Verification items for the finished model (mm, model axes). A direction names the side the tool comes from. Give positions to 0.01 mm unless a question says otherwise; leave off trailing zeros. Write each loop counter-clockwise with the first axis right and the second up, starting at its lowest first coordinate (ties: lowest second). Pieces come first, ordered by that corner, then holes. Notation, with made-up numbers: (13.25, -21) - (21.25, -21) arc R4 ccw to (21.25, -14) - close; hole circle Ø4 at (60.5, 33.5). An arc over 180 degrees is marked (long way). Answer as a JSON object with one key per item and string values. Group by question number.
Item 1: Sectioned sample at D-D, the plane y = 98.5. Record the boundary of the cut face in (x, z), and give its area (3 significant figures).
Item 2: Draft check along X on faces 5 (the face through (52, 207, -25)), 6 (the face through (-17.367, 90.897, -2.1)), 7 (the face through (100, 93, 1)). Enter one of: +X half, -X half, draft (parallel to the pull), parting line (faces both ways), or undercut.
Item 3: Sectioned sample at B-B, the plane y = 50.5. Record the boundary of the cut face in (x, z).
Item 4: Sectioned sample at C-C, the plane x = 55. Record the boundary of the cut face in (y, z), and give its area (3 significant figures).
Item 5: Tool access check on faces 1 (the face through (-94, 95, -65)), 2 (the face through (94, 95, 65)), 3 (the face through (52, 208, 25)), 4 (the face through (79, 57, -40)). Record the directions out of +Z, -Z, +X, -X, +Y, -Y that give a thin tool (end or side, any length) a straight path to the whole face; none if there is none.
Item 6: Go/stop test with flat-tipped pins: pin 1 (7.5 mm diameter, centred on y = 204, z = 51.5, fed in from -X); pin 2 (12.5 mm diameter, centred on x = -44.5, y = 204.5, fed in from +Z); pin 3 (23 mm diameter, centred on x = -87.5, y = 65, fed in from +Z); pin 4 (2 mm diameter, centred on x = -3.5, z = 119, fed in from +Y). Record where each tip stops, or that it passes through.
Item 7: Sectioned sample at A-A, the plane z = -46.5. Record the boundary of the cut face in (x, y), and give its area (3 significant figures).
Item 8: Scan lines: line 1 along Y through (x, z) = (43.5, -29.5); line 2 along Y through (x, z) = (89.5, -36); line 3 along Z through (x, y) = (-91.5, 95). Record each from-to range of solid material in increasing order. Write a range as [from, to].
```python
from build123d import *

# Parameters (mm, degrees)
INCLINED_BASE_BLOCK_DEPTH           = 100
FRONT_NOTCH_CUT_DEPTH               = 285.429253067
FRONT_NOTCH_CUT_DEPTH_BACK          = 285.429253067
FRONT_NOTCH_SKETCH_OUTSIDE_W        = 286.474
FRONT_NOTCH_SKETCH_OUTSIDE_H        = 306.474
TOP_RECESS_CUT_DEPTH                = 285.429253067
TOP_RECESS_CUT_DEPTH_BACK           = 285.429253067
FRONT_FRAME_BOSS_DEPTH              = 65
TOP_CROSS_SLOT_CUT_80X80_DEPTH      = 334.016516107
TOP_CROSS_SLOT_CUT_80X80_DEPTH_BACK = 334.016516107
TOP_CROSS_SLOT_SKETCH_W             = 80
TOP_CROSS_SLOT_SKETCH_H             = 80


with BuildPart() as part:
    # Base Profile Sketch → Inclined Base Block (new, symmetric)
    with BuildSketch(Plane(origin=(0, 0, 0), x_dir=(0, 0, -1), z_dir=(1, 0, 0))):
        Polygon((-150, 0), (-80, 220), (-25, 220), (-25, 195), (25, 195), (25, 220), (80, 220), (150, 0), align=None)
    extrude(amount=INCLINED_BASE_BLOCK_DEPTH, both=True)

    # Front Notch Sketch outside → Front Notch Cut (cut, two sides: drawn at the far end of the back side and taken through both)
    with BuildSketch(Plane.XY.offset(-FRONT_NOTCH_CUT_DEPTH_BACK)):
        with Locations((0, 110)):
            Rectangle(FRONT_NOTCH_SKETCH_OUTSIDE_W, FRONT_NOTCH_SKETCH_OUTSIDE_H)
        Polygon((-100, 0), (-65, 220), (-35, 220), (-35, 195), (35, 195), (35, 220), (65, 220), (100, 0), align=None, mode=Mode.SUBTRACT)
    extrude(amount=FRONT_NOTCH_CUT_DEPTH + FRONT_NOTCH_CUT_DEPTH_BACK, mode=Mode.SUBTRACT)

    # Top Recess Sketch → Top Recess Cut (cut, two sides: drawn at the far end of the back side and taken through both)
    with BuildSketch(Plane.XY.offset(-TOP_RECESS_CUT_DEPTH_BACK)):
        Polygon((-100, 0), (0, 110), (100, 0), align=None)
    extrude(amount=TOP_RECESS_CUT_DEPTH + TOP_RECESS_CUT_DEPTH_BACK, mode=Mode.SUBTRACT)

    # Front Frame Sketch → Front Frame Boss (add, symmetric)
    with BuildSketch(Plane.XY):
        Polygon((100, 0), (100, 130), (79.318181818, 130), align=None)
    front_frame_boss = extrude(amount=FRONT_FRAME_BOSS_DEPTH, both=True)

    # Front Frame Mirror: Front Frame Boss across plane
    add(front_frame_boss.mirror(Plane(origin=(0, 0, 0), x_dir=(0, 0, 1), z_dir=(1, 0, 0))))

    # Top Cross Slot Sketch → Top Cross Slot Cut 80x80 (cut, two sides: drawn at the far end of the back side and taken through both)
    with BuildSketch(Plane(origin=(100, 0, 0), x_dir=(0, 0, -1), z_dir=(1, 0, 0)).offset(-TOP_CROSS_SLOT_CUT_80X80_DEPTH_BACK)):
        with Locations((0, 40)):
            Rectangle(TOP_CROSS_SLOT_SKETCH_W, TOP_CROSS_SLOT_SKETCH_H)
    extrude(amount=TOP_CROSS_SLOT_CUT_80X80_DEPTH + TOP_CROSS_SLOT_CUT_80X80_DEPTH_BACK, mode=Mode.SUBTRACT)


solid = part.part
```
Geometry check:
{
 "1": {"outline": "(-100, -65) - (-84.33, -65) - (-84.33, -118.66) - (-10.45, -118.66) - (-10.45, 118.66) - (-84.33, 118.66) - (-84.33, 65) - (-100, 65) - close; (10.45, -118.66) - (84.33, -118.66) - (84.33, -65) - (100, -65) - (100, 65) - (84.33, 65) - (84.33, 118.66) - (10.45, 118.66) - close", "area": "39,100 mm^2"},
 "2": {"face 5": "draft", "face 6": "undercut", "face 7": "+X half"},
 "3": {"outline": "(-100, -65) - (-91.97, -65) - (-91.97, -133.93) - (-54.09, -133.93) - (-54.09, -40) - (-100, -40) - close; (-100, 40) - (-54.09, 40) - (-54.09, 133.93) - (-91.97, 133.93) - (-91.97, 65) - (-100, 65) - close; (54.09, -133.93) - (91.97, -133.93) - (91.97, -65) - (100, -65) - (100, -40) - (54.09, -40) - close; (54.09, 40) - (100, 40) - (100, 65) - (91.97, 65) - (91.97, 133.93) - (54.09, 133.93) - close"},
 "4": {"outline": "(49.5, -134.25) - (220, -80) - (220, -25) - (195, -25) - (195, 25) - (220, 25) - (220, 80) - (49.5, 134.25) - (49.5, 40) - (80, 40) - (80, -40) - (49.5, -40) - close", "area": "32,800 mm^2"},
 "5": {"face 1": "-Z, -X, +Y", "face 2": "+Z, +X, +Y", "face 3": "+X, -X, +Y", "face 4": "+X, -X, -Y"},
 "6": {"pin 1": "x = -68.14", "pin 2": "z = 86.92", "pin 3": "z = 132.98", "pin 4": "through"},
 "7": {"outline": "(-100, 0) - (0, 110) - (100, 0) - (100, 130) - (79.32, 130) - (65, 220) - (35, 220) - (35, 195) - (-35, 195) - (-35, 220) - (-65, 220) - (-79.32, 130) - (-100, 130) - close", "area": "26,200 mm^2"},
 "8": {"line 1": "[80, 220]", "line 2": "[80, 130]", "line 3": "[-65, 65]"}
}
